from build123d import *

# Parameters (mm, degrees)
BOSS_EXTRUDE1_DEPTH  = 10
LPATTERN1_COUNT      = 2
LPATTERN1_PITCH      = 47
LPATTERN1_COUNT_DIR2 = 2
LPATTERN1_PITCH_DIR2 = 47
LPATTERN2_COUNT      = 2
LPATTERN2_PITCH      = 47
LPATTERN2_COUNT_DIR2 = 2
LPATTERN2_PITCH_DIR2 = 86


with BuildPart() as part:
    # Sketch1 → Boss-Extrude1 (new body)
    with BuildSketch(Plane(origin=(0, 0, 0), x_dir=(0, 0, -1), z_dir=(1, 0, 0))):
        with BuildLine():
            Line((-30.5, -52), (30.5, -52))
            ThreePointArc((30.5, -52), (31.914213562, -51.414213562), (32.5, -50))
            Line((32.5, -50), (32.5, 50))
            ThreePointArc((32.5, 50), (31.914213562, 51.414213562), (30.5, 52))
            Line((30.5, 52), (-30.5, 52))
            ThreePointArc((-30.5, 52), (-31.914213562, 51.414213562), (-32.5, 50))
            Line((-32.5, 50), (-32.5, -50))
            ThreePointArc((-32.5, -50), (-31.914213562, -51.414213562), (-30.5, -52))
        make_face()
    extrude(amount=BOSS_EXTRUDE1_DEPTH)

    # Sketch2 → Cut-Revolve1 (revolve, cut)
    with BuildSketch(Plane(origin=(0, 0, 0), x_dir=(1, 0, 0), z_dir=(0, 1, 0))):
        Polygon((10, 0), (10, -19.65), (9.5, -19.15), (0.5, -19.15), (0, -19.65), (0, 0), align=None)
    revolve(axis=Axis((0, 0, 0), (1, 0, 0)), mode=Mode.SUBTRACT)

    # Sketch3 → Cut-Revolve2 (revolve, cut)
    with BuildSketch(Plane(origin=(0, -23.5, 0), x_dir=(1, 0, 0), z_dir=(0, 1, 0))):
        Polygon((10, 23.5), (10, 20.25), (6.5, 20.25), (6.5, 18.25), (0.5, 18.25), (0, 17.75), (0, 23.5), align=None)
    cut_revolve2 = revolve(axis=Axis((0, -23.5, -23.5), (1, 0, 0)), mode=Mode.SUBTRACT)

    # LPattern1: Cut-Revolve2 2 × 2
    with Locations(*[(0, i * LPATTERN1_PITCH, j * LPATTERN1_PITCH_DIR2) for i in range(LPATTERN1_COUNT) for j in range(LPATTERN1_COUNT_DIR2) if (i, j) != (0, 0)]):
        add(cut_revolve2, mode=Mode.SUBTRACT)

    # Sketch5 → Cut-Revolve3 (revolve, cut)
    with BuildSketch(Plane(origin=(0, -43, 0), x_dir=(1, 0, 0), z_dir=(0, 1, 0))):
        Polygon((0, -23.5), (0, -18.5), (0.5, -19), (10, -19), (10, -23.5), align=None)
    cut_revolve3 = revolve(axis=Axis((10, -43, 23.5), (-1, 0, 0)), mode=Mode.SUBTRACT)

    # LPattern2: Cut-Revolve3 2 × 2
    with Locations(*[(0, j * LPATTERN2_PITCH_DIR2, -i * LPATTERN2_PITCH) for i in range(LPATTERN2_COUNT) for j in range(LPATTERN2_COUNT_DIR2) if (i, j) != (0, 0)]):
        add(cut_revolve3, mode=Mode.SUBTRACT)


solid = part.part
Could you check a few things on this model? Use its own coordinates, in mm. A direction names the side the tool comes from. Coordinates: 2 decimals unless noted, no trailing zeros. Loops run counter-clockwise (first coordinate to the right, second up) from the corner with the lowest first, then second, coordinate; pieces in that order, holes last.
1. For faces 1 (the face through (6.5, -21, -21)), 2 (the face through (8.226, 25.478, -26.079)), which set-ups out of +Z, -Z, +X, -X, +Y, -Y let a thin tool reach every point of the face, with its end or its side?
2. I need wall thicknesses on L1, parallel to Z at x = 7.25, y = -23.5; L2, parallel to Z at x = 1.75, y = -43; L3, parallel to Y at x = 5.05, z = 23.5. Which ranges of each line are inside material? Lowest first, please.
3. Imagine slicing it at D-D (y = -23.5). Please give me the cut outline in (x, z).
4. For P1, Ø3, axis at y = -26, z = 21.5, coming from the -X side, with a flat end and sliding along its axis, tell me the tip position at first contact or that it passes through.
5. We'd pull the mould along Y, two halves only. Please class faces 3 (the face through (4.93, -51.4, 31.93)), 4 (the face through (4.94, 11.65, -15.2)), 5 (the face through (5, -1, -32.5)): released by +Y, released by -Y, zero draft, split by the parting line, or undercut.
6. Imagine slicing it at C-C (z = 0). Please give me the cut outline in (x, y), and give its area (4 significant figures).
7. Imagine slicing it at B-B (x = 5.25). Give the number of separate pieces and of enclosed holes in the cut face, and give its area (3 significant figures).
8. Imagine slicing it at A-A (y = 0). Please give me the cut outline in (x, z).
Computed values:
1. face 1: -X
1. face 2: +X, -X
2. L1: z = -32.5 to -26.75, -20.25 to 20.25, 26.75 to 32.5
2. L2: z = -32.5 to -28, -19 to 19, 28 to 32.5
2. L3: y = -52 to -47.5, -38.5 to -28.75, -18.25 to 18.25, 28.75 to 38.5, 47.5 to 52
3. outline: (0, -32.5) - (10, -32.5) - (10, -26.75) - (6.5, -26.75) - (6.5, -28.75) - (0.5, -28.75) - (0, -29.25) - close; (0, -17.75) - (0.5, -18.25) - (6.5, -18.25) - (6.5, -20.25) - (10, -20.25) - (10, 20.25) - (6.5, 20.25) - (6.5, 18.25) - (0.5, 18.25) - (0, 17.75) - close; (0, 29.25) - (0.5, 28.75) - (6.5, 28.75) - (6.5, 26.75) - (10, 26.75) - (10, 32.5) - (0, 32.5) - close
4. P1: stops at x = 6.5
5. face 3: released by -Y
5. face 4: undercut
5. face 5: zero draft
6. outline: (0, -52) - (10, -52) - (10, -19.65) - (9.5, -19.15) - (0.5, -19.15) - (0, -19.65) - close; (0, 19.65) - (0.5, 19.15) - (9.5, 19.15) - (10, 19.65) - (10, 52) - (0, 52) - close
6. area: 656.5 mm2
7. separate pieces: 1
7. enclosed holes: 9
7. area: 5,000 mm2
8. outline: (0, -32.5) - (10, -32.5) - (10, -19.65) - (9.5, -19.15) - (0.5, -19.15) - (0, -19.65) - close; (0, 19.65) - (0.5, 19.15) - (9.5, 19.15) - (10, 19.65) - (10, 32.5) - (0, 32.5) - close
